Part model, mm, in its own coordinate system. Round coordinates to 2 decimals unless told otherwise and drop trailing zeros. Write each loop counter-clockwise with the first axis right and the second up, starting at its lowest first coordinate (ties: lowest second). Pieces come first, ordered by that corner, then holes. Notation, with made-up numbers: M 60,69 L 104,69 A17 cw 104,80 Z; hole C 60,-20 d2. An arc over 180 degrees is marked long. Use a Markdown table: item, result. Add a question column.
1) Slice it at B-B on y = 107.5. Write the cut outline in (x, z), plus the area to 3 significant figures.
2) Slice it at C-C on y = 47. Write the cut outline in (x, z), plus the area to 3 significant figures.
3) Drop flat-ended pins along their axis: P1, Ø3, axis at x = 1, y = 46, coming from the -Z side; P2, Ø2.5, axis at y = 107.5, z = 0, coming from the +X side. Give the stop position or say it passes through.
4) Slice it at A-A on z = 0. Write the cut outline in (x, y).
5) Wall check: probe 1 along Y at (x, z) = (-0.05, 0); probe 2 along X at (y, z) = (24, 2.25); probe 3 along Z at (x, y) = (1.1, 107.5). Give the ranges that are in metal, low to high.
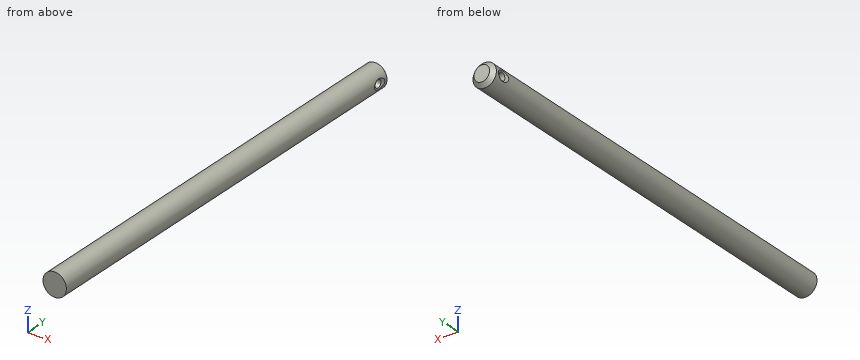
```python
from build123d import *

# Parameters (mm, degrees)
SKETCH1_R               = 3
BOSS_EXTRUDE1_DEPTH     = 111
CUT_EXTRUDE1_DEPTH      = 112.081051489
CUT_EXTRUDE1_DEPTH_BACK = 112.081051489
SKETCH2_R               = 1
CHAMFER3_SIZE           = 1


with BuildPart() as part:
    # Sketch1 → Boss-Extrude1 (new body)
    with BuildSketch(Plane(origin=(0, 0, 0), x_dir=(1, 0, 0), z_dir=(0, 1, 0))):
        with Locations(Location((0, 0, 0), (0, 0, 270))):
            Circle(SKETCH1_R)
    extrude(amount=BOSS_EXTRUDE1_DEPTH)

    # Sketch2 → Cut-Extrude1 (cut, two sides: drawn at the far end of the back side and taken through both)
    with BuildSketch(Plane(origin=(0, 0, 0), x_dir=(0, 0, -1), z_dir=(1, 0, 0)).offset(-CUT_EXTRUDE1_DEPTH_BACK)):
        with Locations((0, 107.5)):
            Circle(SKETCH2_R)
    extrude(amount=CUT_EXTRUDE1_DEPTH + CUT_EXTRUDE1_DEPTH_BACK, mode=Mode.SUBTRACT)

    # Cut-Extrude2 cone 1 section (through the dimple's axis) → Cut-Extrude2 (revolve, cut)
    with BuildSketch(Plane(origin=(3, 107.5, 0), x_dir=(0, 0, -1), z_dir=(0, 1, 0))):
        Polygon((0, 0), (1.75, 0), (0, 1.010362971), align=None)
    cut_extrude2 = revolve(axis=Axis((3, 107.5, 0), (-1, 0, 0)), mode=Mode.SUBTRACT)

    # Mirror1: Cut-Extrude2 across plane
    add(cut_extrude2.mirror(Plane(origin=(0, 0, 0), x_dir=(0, 0, 1), z_dir=(1, 0, 0))), mode=Mode.SUBTRACT)

    # Chamfer3
    chamfer3_edges = [part.edges().sort_by_distance(p)[0] for p in [
        (0, 111, -3),
    ]]
    chamfer(chamfer3_edges, length=CHAMFER3_SIZE)


solid = part.part
```
Entries:
| question | item | result |
|---|---|---|
| 1 | outline | M -2.72,-1.27 A3 ccw 2.72,-1.27 L 2.57,-1 L -2.57,-1 Z; M -2.72,1.27 L -2.57,1 L 2.57,1 L 2.72,1.27 A3 ccw Z |
| 1 | area | 16.4 mm^2 |
| 2 | outline | C 0,0 d6 |
| 2 | area | 28.3 mm^2 |
| 3 | P1 | stops at z = -3 |
| 3 | P2 | stops at x = 2.71 |
| 4 | outline | M -3,0 L 3,0 L 3,105.75 L 2.57,106.5 L -2.57,106.5 L -3,105.75 Z; M -3,109.25 L -2.57,108.5 L 2.57,108.5 L 3,109.25 L 3,110 L 2,111 L -2,111 L -3,110 Z |
| 5 | probe 1 | y = 0 to 106.5, 108.5 to 111 |
| 5 | probe 2 | x = -1.98 to 1.98 |
| 5 | probe 3 | z = -2.79 to -1, 1 to 2.79 |
